Could you check a few things on this drawing? It's one solid part, dimensions in mm from its lowest x, y, z. A direction names the side the tool comes from. Give positions to 0.01 mm unless a question says otherwise; leave off trailing zeros. Loops run counter-clockwise (first coordinate to the right, second up) from the corner with the lowest first, then second, coordinate; pieces in that order, holes last. Notation, with made-up numbers: M 66,23.25 L 89,23.25 A19 cw 89,51.25 Z; hole C 14,62 d2. An arc over 180 degrees is marked long. Return JSON: item names as keys, results as strings. Group by question number.
1. For pin 1 (2 mm diameter, centred on x = 26.5, z = 18, fed in from -Y); pin 2 (6 mm diameter, centred on x = 55, y = 22, fed in from +Z); pin 3 (10 mm diameter, centred on x = 57.5, z = 21, fed in from -Y), each with a flat end and sliding along its axis, tell me the tip position at first contact or that it passes through.
2. If we section it at D-D (x = 92): Write out the boundary of the cut face in (y, z), plus the area to 3 significant figures.
3. If we section it at C-C (x = 7): Write out the boundary of the cut face in (y, z), plus the area to 3 significant figures.
4. Please list where these lines run through material, in increasing order: line 1 (X direction, y = 16, z = 16); line 2 (Y direction, x = 7, z = 16.5); line 3 (X direction, y = 4.5, z = 13.5).
5. If we section it at A-A (y = 16): Write out the boundary of the cut face in (x, z), plus the area to 3 significant figures.
6. For the marked faces 1 and 2, which set-ups out of +Z, -Z, +X, -X, +Y, -Y let a thin tool reach every point of the face, with its end or its side?
7. If we section it at B-B (z = 16): Write out the boundary of the cut face in (x, y).
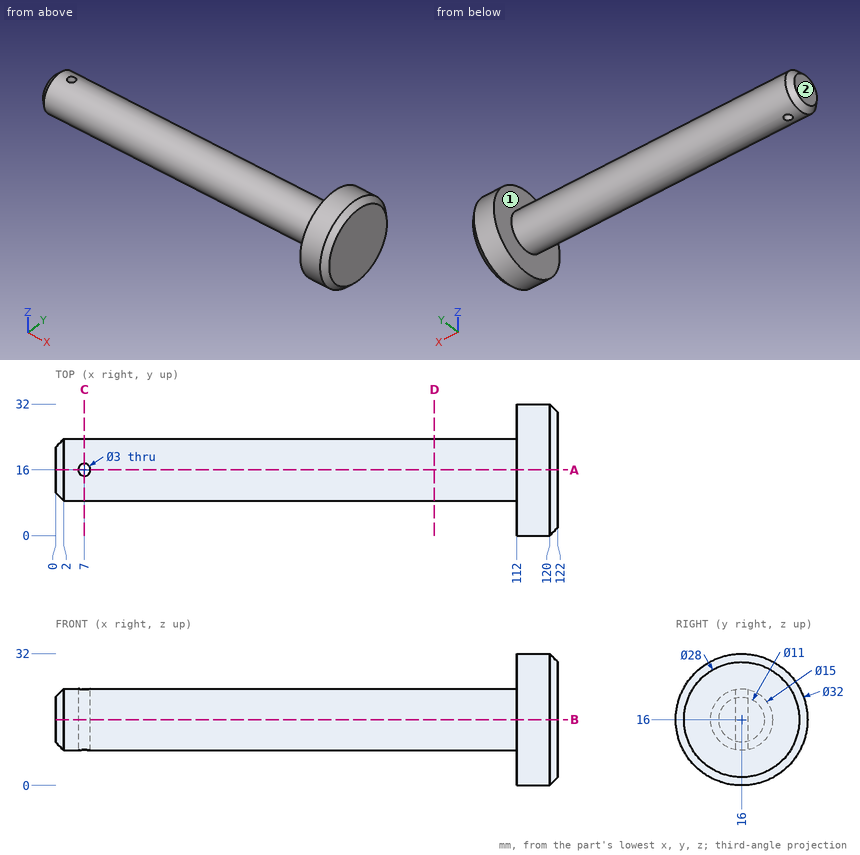
Answer:
{
 "1": {"pin 1": "stops at y = 8.57", "pin 2": "stops at z = 22.87", "pin 3": "stops at y = 8.5"},
 "2": {"outline": "C 16,16 d15", "area": "177 mm²"},
 "3": {"outline": "M 14.5,8.65 L 14.5,23.35 A7.5 ccw Z; M 17.5,8.65 A7.5 ccw 17.5,23.35 Z", "area": "132 mm²"},
 "4": {"line 1": "x = 0 to 5.5, 8.5 to 122", "line 2": "y = 8.52 to 14.5, 17.5 to 23.48", "line 3": "x = 112 to 122"},
 "5": {"outline": "M 0,10.5 L 2,8.5 L 5.5,8.5 L 5.5,23.5 L 2,23.5 L 0,21.5 Z; M 8.5,8.5 L 112,8.5 L 112,0 L 120,0 L 122,2 L 122,30 L 120,32 L 112,32 L 112,23.5 L 8.5,23.5 Z", "area": "1,950 mm²"},
 "6": {"face 1": "-X", "face 2": "+Z, -Z, -X, +Y, -Y"},
 "7": {"outline": "M 0,10.5 L 2,8.5 L 112,8.5 L 112,0 L 120,0 L 122,2 L 122,30 L 120,32 L 112,32 L 112,23.5 L 2,23.5 L 0,21.5 Z; hole C 7,16 d3"}
}
